Verification items for the finished model (mm, model axes). Face numbers are marked on the shaded views. A direction names the side the tool comes from. Round coordinates to 2 decimals unless told otherwise and drop trailing zeros. Write each loop counter-clockwise with the first axis right and the second up, starting at its lowest first coordinate (ties: lowest second). Pieces come first, ordered by that corner, then holes. Notation, with made-up numbers: M -35,-7 L 15,-7 A19 cw 15,16 Z; hole C 59,46.25 d5. An arc over 180 degrees is marked long. One line per item, written item: value. Start each with the question number.
Item 1: Draft check along X on the marked faces 3, 4 and 5. Enter one of: +X half, -X half, draft (parallel to the pull), parting line (faces both ways), or undercut.
Item 2: Gauge pin test, flat ends, axial feed: pin 1 (4.5 mm diameter, centred on x = 0, y = -10, fed in from -Z); pin 2 (1 mm diameter, centred on x = -1, y = 5, fed in from +Z); pin 3 (3 mm diameter, centred on x = 0, y = 0, fed in from +Z); pin 4 (12 mm diameter, centred on x = -4.5, z = 16.5, fed in from -Y). Record the tip position at first contact, or that the pin passes through.
Item 3: Tool access check on the marked faces 1 and 2. Record the directions out of +Z, -Z, +X, -X, +Y, -Y that give a thin tool (end or side, any length) a straight path to the whole face; none if there is none.
Item 4: Section check A-A, the plane z = -1. Record the cut outline in (x, y).
Item 5: Thickness scan on probe 1 along X at (y, z) = (0, 15.25); probe 2 along Z at (x, y) = (7.5, -2.25). Record the ranges inside material, lowest first. Write a range as from..to.
Item 6: Section check B-B, the plane z = 11.25. Record the cut outline in (x, y), then the cut area to 3 significant figures.
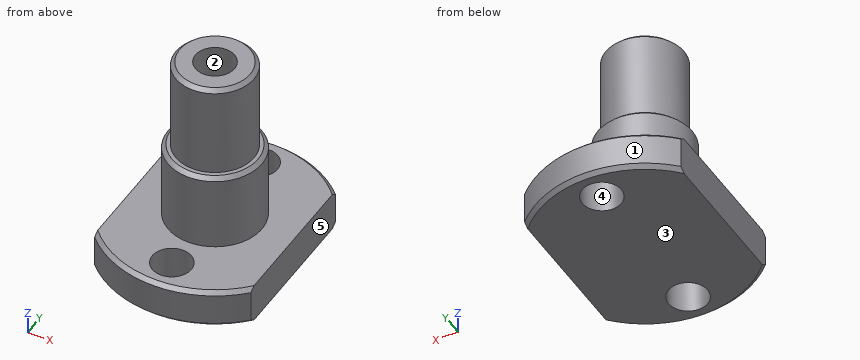
from build123d import *

# Parameters (mm, degrees)
SKETCH_1_R                = 5
EXTRUDE_1_DEPTH           = 22
SKETCH_2_R                = 6
EXTRUDE_2_DEPTH           = 10
SKETCH_3_R                = 14
EXTRUDE_3_DEPTH           = 5
SKETCH_4_OUTSIDE_W        = 39.586
SKETCH_4_OUTSIDE_H        = 39.586
SKETCH_4_OUTSIDE_W_2      = 20
SKETCH_4_OUTSIDE_H_2      = 37.741501618
CUT_EXTRUDE_1_DEPTH       = 5
HOLE_WIZARD_5_0_5_1_D     = 5
HOLE_WIZARD_5_0_5_1_DEPTH = 20
HOLE_WIZARD_5_0_5_1_TIP   = 1.502151548
HOLE_WIZARD_M6_1_D        = 5
HOLE_WIZARD_M6_1_DEPTH    = 15
HOLE_WIZARD_M6_1_TIP      = 1.502151548
CHAMFER_1_SIZE            = 0.5
CHAMFER_2_SIZE            = 0.5


with BuildPart() as part:
    # 草图1 → 凸台-拉伸1 (new body)
    with BuildSketch(Plane.XY):
        Circle(SKETCH_1_R)
    extrude(amount=EXTRUDE_1_DEPTH)

    # 草图2 → 凸台-拉伸2 (add)
    with BuildSketch(Plane(origin=(0, 0, 0), x_dir=(-1, 0, 0), z_dir=(0, 0, -1))):
        Circle(SKETCH_2_R)
    extrude(amount=-EXTRUDE_2_DEPTH)

    # 草图3 → 凸台-拉伸3 (add)
    with BuildSketch(Plane(origin=(0, 0, 0), x_dir=(-1, 0, 0), z_dir=(0, 0, -1))):
        Circle(SKETCH_3_R)
    extrude(amount=EXTRUDE_3_DEPTH)

    # 草图4 outside → 切除-拉伸1 (cut)
    with BuildSketch(Plane(origin=(0, 0, -5), x_dir=(-1, 0, 0), z_dir=(0, 0, -1))):
        Rectangle(SKETCH_4_OUTSIDE_W, SKETCH_4_OUTSIDE_H)
        with Locations((0, -0.226902815)):
            Rectangle(SKETCH_4_OUTSIDE_W_2, SKETCH_4_OUTSIDE_H_2, mode=Mode.SUBTRACT)
    extrude(amount=-CUT_EXTRUDE_1_DEPTH, mode=Mode.SUBTRACT)

    # Ø5.0 (5) 直径孔1
    with Locations(Plane.XY):
        with Locations((0, 10), (0, -10)):
            Hole(HOLE_WIZARD_5_0_5_1_D / 2, depth=HOLE_WIZARD_5_0_5_1_DEPTH)
            with Locations((0, 0, -(HOLE_WIZARD_5_0_5_1_DEPTH + HOLE_WIZARD_5_0_5_1_TIP / 2))):  # 118° drill point
                Cone(0, HOLE_WIZARD_5_0_5_1_D / 2, HOLE_WIZARD_5_0_5_1_TIP, mode=Mode.SUBTRACT)

    # M6 螺纹孔1
    with Locations(Plane.XY.offset(22)):
        with Locations((0, 0)):
            Hole(HOLE_WIZARD_M6_1_D / 2, depth=HOLE_WIZARD_M6_1_DEPTH)
            with Locations((0, 0, -(HOLE_WIZARD_M6_1_DEPTH + HOLE_WIZARD_M6_1_TIP / 2))):  # 118° drill point
                Cone(0, HOLE_WIZARD_M6_1_D / 2, HOLE_WIZARD_M6_1_TIP, mode=Mode.SUBTRACT)

    # 倒角1
    chamfer_1_edges = [part.edges().sort_by_distance(p)[0] for p in [
        (-5, 0, 22),
        (6, 0, 10),
    ]]
    chamfer(chamfer_1_edges, length=CHAMFER_1_SIZE)

    # 倒角2
    chamfer_2_edges = [part.edges().sort_by_distance(p)[0] for p in [
        (0, 14, 0),
        (0, 14, -5),
        (0, -14, 0),
        (0, -14, -5),
    ]]
    chamfer(chamfer_2_edges, length=CHAMFER_2_SIZE)


solid = part.part
Response values:
1. face 3: draft
1. face 4: undercut
1. face 5: +X half
2. pin 1: passes through
2. pin 2: stops at z = 21.9
2. pin 3: stops at z = 6.4
2. pin 4: stops at y = -5
3. face 1: +Z, -Z, +Y
3. face 2: +Z
4. outline: M -10,-9.8 A14 ccw 10,-9.8 L 10,9.8 A14 ccw -10,9.8 Z; hole C 0,-10 d5; hole C 0,10 d5
5. probe 1: x = -5..-2.5, 2.5..5
5. probe 2: z = -5..0
6. outline: C 0,0 d10; hole C 0,0 d5
6. area: 58.9 mm2
